Input: part model. Units: mm. Frame: model coordinates. Round coordinates to 2 decimals unless told otherwise and drop trailing zeros. Loops run counter-clockwise (first coordinate to the right, second up) from the corner with the lowest first, then second, coordinate; pieces in that order, holes last. Notation, with made-up numbers: M 86.25,54.5 L 127.25,54.5 A31 ccw 127.25,91.5 Z; hole C 70.25,-34 d3. An arc over 180 degrees is marked long. Return JSON: item names as keys, results as strings. Group by question number.
1) Contact query for flat-ended pins moving along their axis: P1, Ø1, axis at x = 0, z = 49.5, coming from the -Y side; P2, Ø8, axis at x = -11, z = 61.5, coming from the -Y side; P3, Ø6, axis at y = -8.5, z = 39, coming from the +X side. Output: stop coordinate, or through.
2) Material intervals for line 1 (Z direction, x = 0, y = 2); line 2 (Z direction, x = -16, y = -10); line 3 (X direction, y = -1, z = 73), sorted ascending. Write a range as from..to.
3) Section C-C (z = 73). Output: boundary loops of the cut face in (x, y).
4) Section B-B (y = 0). Output: boundary loops of the cut face in (x, z).
5) Section D-D (x = -24). Output: boundary loops of the cut face in (y, z), plus the area to 3 significant figures.
6) Section A-A (x = 0). Output: boundary loops of the cut face in (y, z).
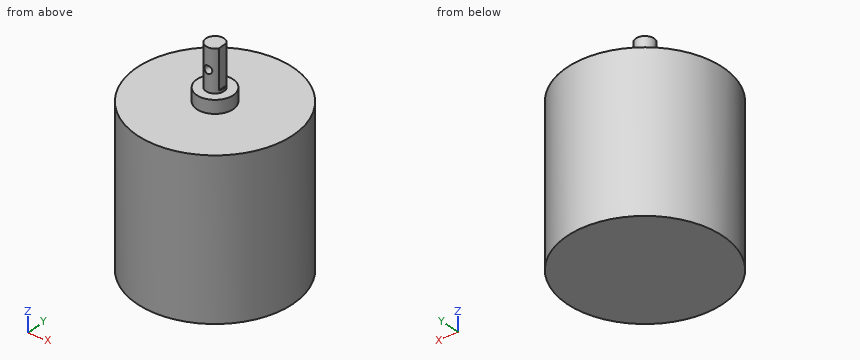
from build123d import *

# Parameters (mm, degrees)
SKETCH_1_R          = 30
EXTRUDE_1_DEPTH     = 60
SKETCH_2_R          = 7
EXTRUDE_2_DEPTH     = 5
SKETCH_3_R          = 3.5
EXTRUDE_3_DEPTH     = 16
CUT_EXTRUDE_START   = -15
CUT_EXTRUDE_1_DEPTH = 15
SKETCH_5_R          = 1.5
CUT_EXTRUDE_2_DEPTH = 7.5


with BuildPart() as part:
    # Sketch 1 → Extrude 1 (new body)
    with BuildSketch(Plane.XY):
        Circle(SKETCH_1_R)
    extrude(amount=EXTRUDE_1_DEPTH)

    # Sketch 2 → Extrude 2 (add)
    with BuildSketch(Plane.XY.offset(60)):
        Circle(SKETCH_2_R)
    extrude(amount=EXTRUDE_2_DEPTH)

    # Sketch 3 → Extrude 3 (add)
    with BuildSketch(Plane.XY.offset(65)):
        Circle(SKETCH_3_R)
    extrude(amount=EXTRUDE_3_DEPTH)

    # Sketch 4 → Cut-Extrude 1 (cut)
    with BuildSketch(Plane.XY.offset(81).offset(CUT_EXTRUDE_START)):
        with BuildLine():
            ThreePointArc((3.5, 0), (3.372684391, 0.935414347), (3, 1.802775638))
            Line((3, 1.802775638), (3, 0))
            Line((3, 0), (3.5, 0))
        make_face()
        with BuildLine():
            Line((3.5, 0), (3, 0))
            Line((3, 0), (3, -1.802775638))
            ThreePointArc((3, -1.802775638), (3.372684391, -0.935414347), (3.5, 0))
        make_face()
    extrude(amount=CUT_EXTRUDE_1_DEPTH, mode=Mode.SUBTRACT)

    # Sketch 5 → Cut-Extrude 2 (cut, symmetric)
    with BuildSketch(Plane(origin=(3, 0, 0), x_dir=(0, 0, -1), z_dir=(0, -1, 0))):
        with Locations((-73, -3)):
            Circle(SKETCH_5_R)
    extrude(amount=CUT_EXTRUDE_2_DEPTH, both=True, mode=Mode.SUBTRACT)


solid = part.part
Returned:
{
 "1": {"P1": "stops at y = -30", "P2": "stops at y = -29.1", "P3": "stops at x = 29.49"},
 "2": {"line 1": "z = 0..71.5, 74.5..81", "line 2": "z = 0..60", "line 3": "x = -3.35..-1.5, 1.5..3"},
 "3": {"outline": "M -1.5,-3.16 L -1.5,3.16 A3.5 ccw Z; M 1.5,-3.16 A3.5 ccw 3,-1.8 L 3,1.8 A3.5 ccw 1.5,3.16 Z"},
 "4": {"outline": "M -30,0 L 30,0 L 30,60 L 7,60 L 7,65 L 3.5,65 L 3.5,66 L 3,66 L 3,81 L -3.5,81 L -3.5,65 L -7,65 L -7,60 L -30,60 Z; hole C 0,73 d3"},
 "5": {"outline": "M -18,0 L 18,0 L 18,60 L -18,60 Z", "area": "2,160 mm^2"},
 "6": {"outline": "M -30,0 L 30,0 L 30,60 L 7,60 L 7,65 L 3.5,65 L 3.5,71.5 L -3.5,71.5 L -3.5,65 L -7,65 L -7,60 L -30,60 Z; M -3.5,74.5 L 3.5,74.5 L 3.5,81 L -3.5,81 Z"}
}
